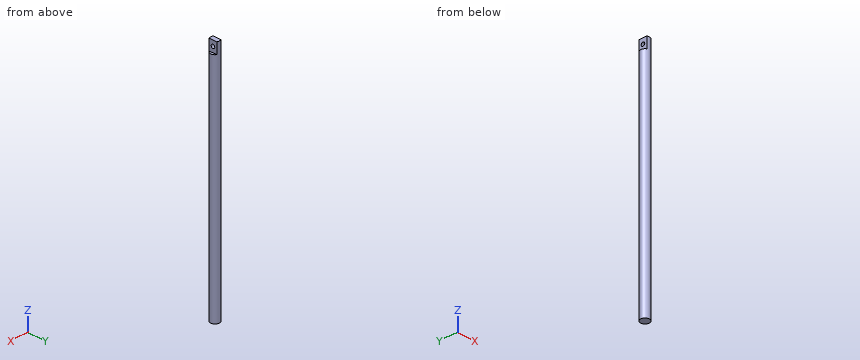
```python
from build123d import *

# Parameters (mm, degrees)
SKETCH1_R               = 20
BOSS_EXTRUDE1_DEPTH     = 1100
CUT_EXTRUDE1_DEPTH      = 1101.363576278
CUT_EXTRUDE1_DEPTH_BACK = 1101.363576278
SKETCH2_W               = 10
SKETCH2_H               = 50
CUT_EXTRUDE2_DEPTH      = 1101.590750461
CUT_EXTRUDE2_DEPTH_BACK = 1101.590750461
SKETCH3_R               = 8.25


with BuildPart() as part:
    # Sketch1 → Boss-Extrude1 (new body)
    with BuildSketch(Plane.XY):
        Circle(SKETCH1_R)
    extrude(amount=BOSS_EXTRUDE1_DEPTH)

    # Sketch2 → Cut-Extrude1 (cut, two sides: drawn at the far end of the back side and taken through both)
    with BuildSketch(Plane(origin=(0, 0, 0), x_dir=(1, 0, 0), z_dir=(0, 1, 0)).offset(-CUT_EXTRUDE1_DEPTH_BACK)):
        with Locations((-15, -1075)):
            Rectangle(SKETCH2_W, SKETCH2_H)
        with Locations((15, -1075)):
            Rectangle(SKETCH2_W, SKETCH2_H)
    extrude(amount=CUT_EXTRUDE1_DEPTH + CUT_EXTRUDE1_DEPTH_BACK, mode=Mode.SUBTRACT)

    # Sketch3 → Cut-Extrude2 (cut, two sides: drawn at the far end of the back side and taken through both)
    with BuildSketch(Plane.ZY.offset(10).offset(-CUT_EXTRUDE2_DEPTH_BACK)):
        with Locations((1075, 0)):
            Circle(SKETCH3_R)
    extrude(amount=CUT_EXTRUDE2_DEPTH + CUT_EXTRUDE2_DEPTH_BACK, mode=Mode.SUBTRACT)


solid = part.part
```
Here's how the part is built. I have some questions about the finished solid (model axes, mm). Round coordinates to 2 decimals unless told otherwise and drop trailing zeros. Write each loop counter-clockwise with the first axis right and the second up, starting at its lowest first coordinate (ties: lowest second). Pieces come first, ordered by that corner, then holes.
Q1. If we section it at C-C on z = 412.5: Write out the boundary of the cut face in (x, y).
Q2. Please list where these lines run through material, in increasing order: probe 1 along Z at (x, y) = (0, 0); probe 2 along X at (y, z) = (1.5, 691.5); probe 3 along Y at (x, z) = (-10, 270).
Q3. Will these pins go through, and if not, where does the flat tip stop? P1, Ø5, axis at x = -7.5, z = 487.5, coming from the +Y side; P2, Ø3, axis at y = 11.5, z = 560, coming from the -X side; P3, Ø17.5, axis at y = 6, z = 1070.5, coming from the +X side.
Q4. If we section it at A-A on y = 0: Write out the boundary of the cut face in (x, z), plus the area to 3 significant figures.
Q5. If we section it at B-B on x = 3: Write out the boundary of the cut face in (y, z).
Answer below:
1. outline: circle Ø40 at (0, 0)
2. probe 1: z = 0 to 1066.75, 1083.25 to 1100
2. probe 2: x = -19.94 to 19.94
2. probe 3: y = -17.32 to 17.32
3. P1: stops at y = 19.36
3. P2: stops at x = -17.32
3. P3: stops at x = 10
4. outline: (-20, 0) - (20, 0) - (20, 1050) - (10, 1050) - (10, 1066.75) - (-10, 1066.75) - (-10, 1050) - (-20, 1050) - close; (-10, 1083.25) - (10, 1083.25) - (10, 1100) - (-10, 1100) - close
4. area: 42,700 mm2
5. outline: (-19.77, 0) - (19.77, 0) - (19.77, 1100) - (-19.77, 1100) - close; hole circle Ø16.5 at (0, 1075)
